from build123d import *

# Parameters (mm, degrees)
SKETCH1_W           = 15
SKETCH1_H           = 15
BOSS_EXTRUDE1_DEPTH = 20
SKETCH5_W           = 2
SKETCH5_H           = 2
CUT_EXTRUDE1_DEPTH  = 18
SKETCH2_R           = 0.9
CUT_EXTRUDE2_DEPTH  = 71
SKETCH6_R           = 1
BOSS_EXTRUDE2_DEPTH = 2
SKETCH7_R           = 0.75
BOSS_EXTRUDE3_DEPTH = 5


with BuildPart() as part:
    # Sketch1 → Boss-Extrude1 (new body)
    with BuildSketch(Plane.XY):
        Rectangle(SKETCH1_W, SKETCH1_H)
    extrude(amount=BOSS_EXTRUDE1_DEPTH)

    # Sketch5 → Cut-Extrude1 (cut)
    with BuildSketch(Plane(origin=(0, 0, 0), x_dir=(-1, 0, 0), z_dir=(0, 0, -1))):
        with Locations((6.5, 6.5)):
            Rectangle(SKETCH5_W, SKETCH5_H)
        with Locations((6.5, -6.5)):
            Rectangle(SKETCH5_W, SKETCH5_H)
        with Locations((-6.5, -6.5)):
            Rectangle(SKETCH5_W, SKETCH5_H)
        with Locations((-6.5, 6.5)):
            Rectangle(SKETCH5_W, SKETCH5_H)
    extrude(amount=-CUT_EXTRUDE1_DEPTH, mode=Mode.SUBTRACT)

    # Sketch2 → Cut-Extrude2 (cut)
    with BuildSketch(Plane.XY.offset(20)):
        with Locations((6.4, 6.4)):
            Circle(SKETCH2_R)
        with Locations((-6.4, 6.4)):
            Circle(SKETCH2_R)
        with Locations((-6.4, -6.4)):
            Circle(SKETCH2_R)
        with Locations((6.4, -6.4)):
            Circle(SKETCH2_R)
    extrude(amount=-CUT_EXTRUDE2_DEPTH, mode=Mode.SUBTRACT)

    # Sketch6 → Boss-Extrude2 (add)
    with BuildSketch(Plane.XY.offset(20)):
        with Locations(Location((0, 0, 0), (0, 0, 180))):
            Circle(SKETCH6_R)
    extrude(amount=BOSS_EXTRUDE2_DEPTH)

    # Sketch7 → Boss-Extrude3 (add)
    with BuildSketch(Plane.XY.offset(22)):
        Circle(SKETCH7_R)
    extrude(amount=BOSS_EXTRUDE3_DEPTH)


solid = part.part
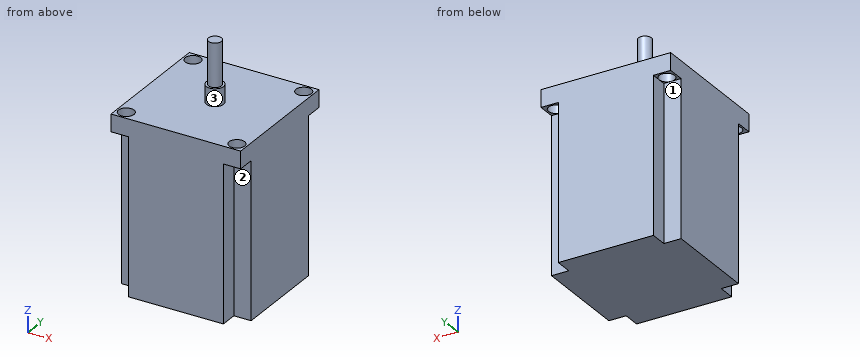
The listing builds one solid part. Answer for the finished solid, in the listing's coordinates (mm). Face numbers are marked on the shaded views. A direction names the side the tool comes from. Round coordinates to 2 decimals unless told otherwise and drop trailing zeros. Write each loop counter-clockwise with the first axis right and the second up, starting at its lowest first coordinate (ties: lowest second). Pieces come first, ordered by that corner, then holes. Notation, with made-up numbers: (-37, -28.75) - (-28, -28.75) arc R24 cw to (-28, 5.25) - close; hole circle Ø5 at (13, -22.5). An arc over 180 degrees is marked (long way). Use one line per item in the form item = value. Start each with the question number.
Item 1: A cutting plane is placed at C-C (y = 3.5). Write down the section's boundary in (x, z), plus the area to 3 significant figures.
Item 2: A cutting plane is placed at D-D (x = -6). Write down the section's boundary in (y, z).
Item 3: Flat-ended cylindrical pins translate along their axes: pin 1 Ø6 at (y, z) = (-3.5, 24) entering from -X; pin 2 Ø1.6 at (x, y) = (-6.5, 6.5) entering from -Z; pin 3 Ø1 at (x, y) = (6.5, -6.5) entering from -Z; pin 4 Ø0.6 at (x, z) = (-7, 5.5) entering from +Y. Find the tip coordinate at first contact, or state that the pin passes through.
Item 4: Find the intervals of material crossed by line 1 (X direction, y = -6.4, z = 19.1); line 2 (Z direction, x = -0.5, y = -6), in increasing order. Write a range as [from, to].
Item 5: A tool of negligible diameter and unlimited length cuts with its end or side. For the marked faces 1, 2 and 3, from which of +Z, -Z, +X, -X, +Y, -Y can it reach the whole face along a straight path? Write none if from no direction.
Item 6: A cutting plane is placed at A-A (x = 0). Write down the section's boundary in (y, z), plus the area to 4 significant figures.
Item 7: A cutting plane is placed at B-B (x = 6.75). Write down the section's boundary in (y, z), plus the area to 3 significant figures.
The answers:
q1.outline = (-7.5, 0) - (7.5, 0) - (7.5, 20) - (-7.5, 20) - close
q1.area = 300 mm^2
q2.outline = (-7.5, 18) - (-7.21, 18) - (-7.21, 20) - (-7.5, 20) - close; (-5.59, 18) - (-5.5, 18) - (-5.5, 0) - (5.5, 0) - (5.5, 18) - (5.59, 18) - (5.59, 20) - (-5.59, 20) - close; (7.21, 18) - (7.5, 18) - (7.5, 20) - (7.21, 20) - close
q3.pin_1 = -0.56
q3.pin_2 = 18
q3.pin_3 = through
q3.pin_4 = 5.5
q4.line_1 = [-7.5, -7.3], [-5.5, 5.5], [7.3, 7.5]
q4.line_2 = [0, 20]
q5.face_1 = -Z, -X, +Y
q5.face_2 = -Z, +X, -Y
q5.face_3 = +Z
q6.outline = (-7.5, 0) - (7.5, 0) - (7.5, 20) - (1, 20) - (1, 22) - (0.75, 22) - (0.75, 27) - (-0.75, 27) - (-0.75, 22) - (-1, 22) - (-1, 20) - (-7.5, 20) - close
q6.area = 311.5 mm^2
q7.outline = (-7.5, 18) - (-7.23, 18) - (-7.23, 20) - (-7.5, 20) - close; (-5.57, 18) - (-5.5, 18) - (-5.5, 0) - (5.5, 0) - (5.5, 18) - (5.57, 18) - (5.57, 20) - (-5.57, 20) - close; (7.23, 18) - (7.5, 18) - (7.5, 20) - (7.23, 20) - close
q7.area = 221 mm^2
